Source: CAD feature listing. Evaluate the final solid. Frame: model axes, mm. Give positions to 0.01 mm unless a question says otherwise; leave off trailing zeros. Order: outer loops, then holes, each group sorted by start corner. A loop starts at its lowest first (then second) coordinate and runs counter-clockwise, first axis right, second up. Notation, with made-up numbers: (-34, 80) - (-23, 80) arc R22 ccw to (-23, 102) - close; hole circle Ø1 at (-18.5, -29). An arc over 180 degrees is marked (long way). Use CSV: the item, a comma, the result in double quotes.
```python
from build123d import *

# Parameters (mm, degrees)
SKETCH_1_R             = 10
EXTRUDE_1_DEPTH        = 445
HOLE_WIZARD_M5_1_D     = 4.2
HOLE_WIZARD_M5_1_DEPTH = 15
HOLE_WIZARD_M5_1_TIP   = 1.2618073
HOLE_WIZARD_M5_2_D     = 4.2
HOLE_WIZARD_M5_2_DEPTH = 15
HOLE_WIZARD_M5_2_TIP   = 1.2618073


with BuildPart() as part:
    # 草图1 → 凸台-拉伸1 (new body)
    with BuildSketch(Plane.XY):
        Circle(SKETCH_1_R)
    extrude(amount=EXTRUDE_1_DEPTH)

    # M5 螺纹孔1
    with Locations(Plane.XY.offset(445)):
        with Locations((0, 0)):
            Hole(HOLE_WIZARD_M5_1_D / 2, depth=HOLE_WIZARD_M5_1_DEPTH)
            with Locations((0, 0, -(HOLE_WIZARD_M5_1_DEPTH + HOLE_WIZARD_M5_1_TIP / 2))):  # 118° drill point
                Cone(0, HOLE_WIZARD_M5_1_D / 2, HOLE_WIZARD_M5_1_TIP, mode=Mode.SUBTRACT)

    # M5 螺纹孔2
    with Locations(Plane(origin=(0, 0, 0), x_dir=(-1, 0, 0), z_dir=(0, 0, -1))):
        with Locations((0, 0)):
            Hole(HOLE_WIZARD_M5_2_D / 2, depth=HOLE_WIZARD_M5_2_DEPTH)
            with Locations((0, 0, -(HOLE_WIZARD_M5_2_DEPTH + HOLE_WIZARD_M5_2_TIP / 2))):  # 118° drill point
                Cone(0, HOLE_WIZARD_M5_2_D / 2, HOLE_WIZARD_M5_2_TIP, mode=Mode.SUBTRACT)


solid = part.part
```
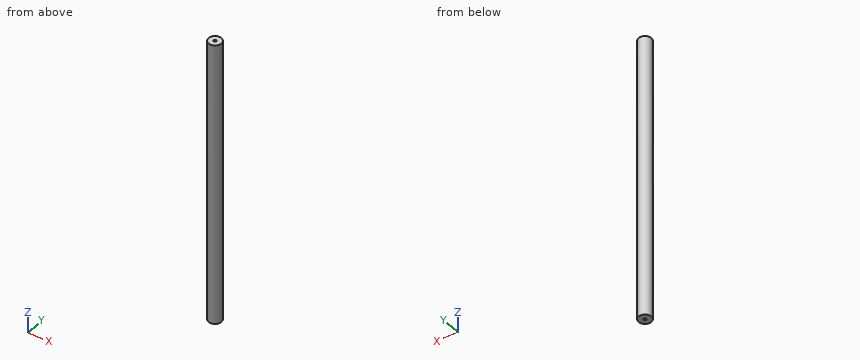
Item 1: First-contact query: pin 1 (6 mm diameter, centred on y = 7, z = 399, fed in from -X); pin 2 (5 mm diameter, centred on x = 8, z = 362, fed in from +Y); pin 3 (2 mm diameter, centred on x = 3, z = 172, fed in from +Y). Flat tips, straight axial feed; report the tip coordinate or a pass-through.
Filled in:
pin 1,"stops at x = -9.17"
pin 2,"stops at y = 8.35"
pin 3,"stops at y = 9.8"
Item 2: Material intervals for line 1 (Y direction, x = 0, z = 433.75); line 2 (Y direction, x = 1.25, z = 213.5); line 3 (Z direction, x = 0, y = 1.25), sorted ascending. Write a range as from..to.
Filled in:
line 1,"y = -10..-2.1, 2.1..10"
line 2,"y = -9.92..9.92"
line 3,"z = 15.51..429.49"
Item 3: Section C-C on y = 7. Return the cut outline in (x, z), then the cut area to 3 significant figures.
Filled in:
outline,"(-7.14, 0) - (7.14, 0) - (7.14, 445) - (-7.14, 445) - close"
area,"6,360 mm2"
Item 4: Section A-A on z = 136.5. Return the cut outline in (x, y), then the cut area to 3 significant figures.
Filled in:
outline,"circle Ø20 at (0, 0)"
area,"314 mm2"
Item 5: Section B-B on x = -6.5. Return the cut outline in (y, z).
Filled in:
outline,"(-7.6, 0) - (7.6, 0) - (7.6, 445) - (-7.6, 445) - close"
